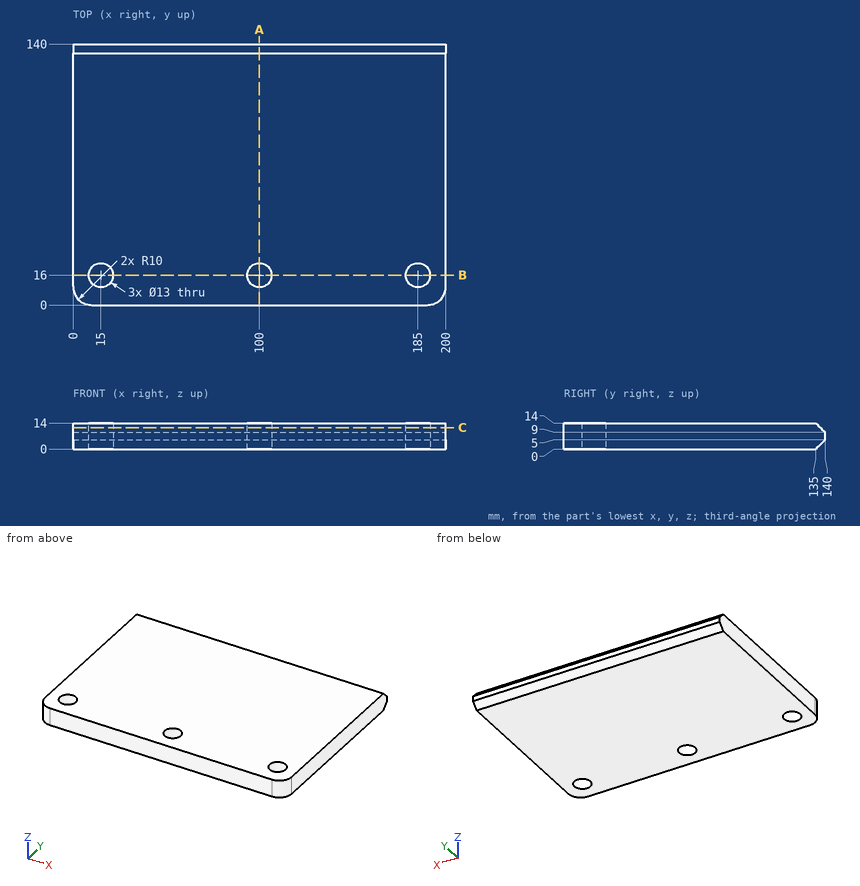
Geometry: see drawing. Coordinates: mm, zero at the bounding-box minimum. Give positions to 0.01 mm unless a question says otherwise; leave off trailing zeros. Order: outer loops, then holes, each group sorted by start corner. A loop starts at its lowest first (then second) coordinate and runs counter-clockwise, first axis right, second up. Notation, with made-up numbers: M -17.75,79 L 34.25,79 A24 cw 34.25,114 Z; hole C -29.5,-34 d7. An arc over 180 degrees is marked long. Answer as a JSON object with one key per item and string values.
1. Cut plane C-C, the plane z = 11.5. Output: boundary loops of the cut face in (x, y).
Result sheet:
{"outline": "M 0,10 A10 ccw 10,0 L 190,0 A10 ccw 200,10 L 200,137.5 L 0,137.5 Z; hole C 15,16 d13; hole C 100,16 d13; hole C 185,16 d13"}
2. Ray query, line 1 (Y direction, x = 100, z = 5); line 2 (X direction, y = 10.5, z = 4.5); line 3 (X direction, y = 17, z = 11.5). Return the intervals inside material, ascending. Write a range as [from, to].
Result sheet:
{"line 1": "[0, 9.5], [22.5, 140]", "line 2": "[0, 11.54], [18.46, 96.54], [103.46, 181.54], [188.46, 200]", "line 3": "[0, 8.58], [21.42, 93.58], [106.42, 178.58], [191.42, 200]"}
3. Cut plane A-A, the plane x = 100. Output: boundary loops of the cut face in (y, z).
Result sheet:
{"outline": "M 0,0 L 9.5,0 L 9.5,14 L 0,14 Z; M 22.5,0 L 135,0 L 140,5 L 140,9 L 135,14 L 22.5,14 Z"}
4. First-contact query: P1, Ø10.5, axis at x = 15, y = 16, coming from the +Z side. Flat tip, straight axial feed; report the tip coordinate or a pass-through.
Result sheet:
{"P1": "through"}
5. Cut plane B-B, the plane y = 16. Output: boundary loops of the cut face in (x, z).
Result sheet:
{"outline": "M 0,0 L 8.5,0 L 8.5,14 L 0,14 Z; M 21.5,0 L 93.5,0 L 93.5,14 L 21.5,14 Z; M 106.5,0 L 178.5,0 L 178.5,14 L 106.5,14 Z; M 191.5,0 L 200,0 L 200,14 L 191.5,14 Z"}
